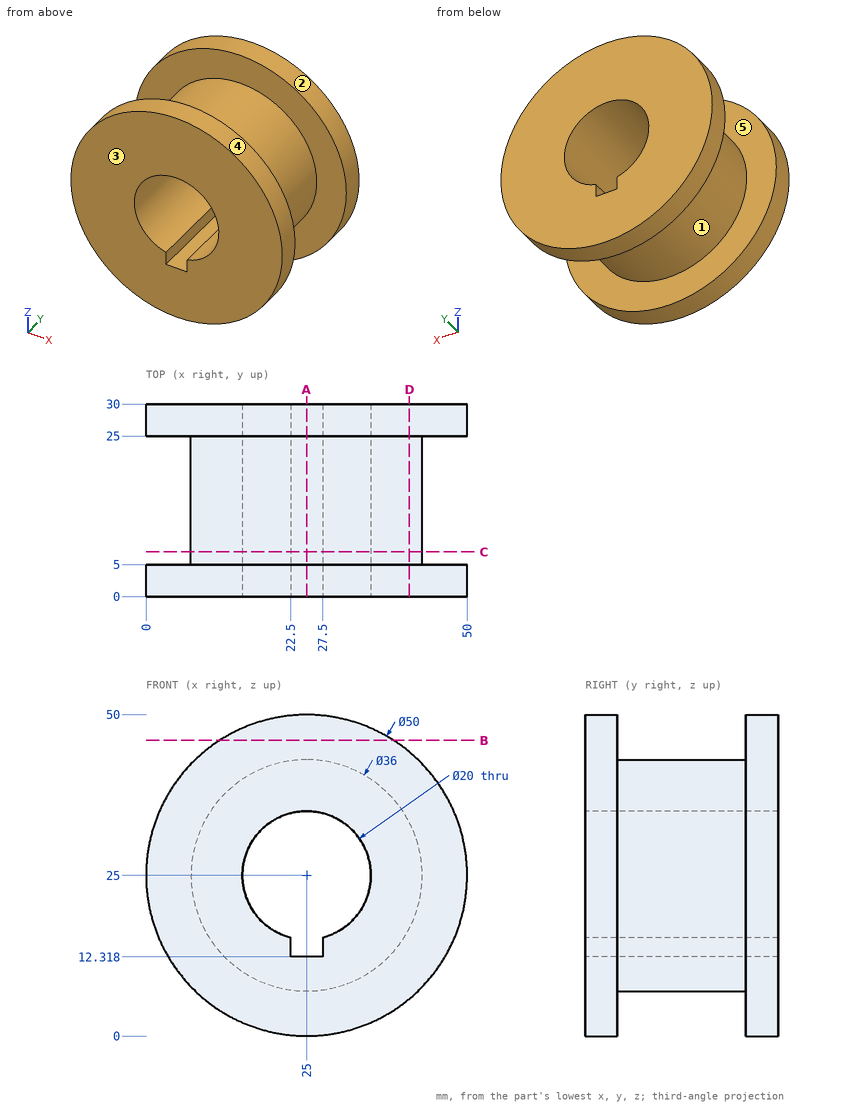
The figure shows three views and two pictorial views of one solid part (mm, origin at its lowest corner). Answer the questions. A direction names the side the tool comes from. Coordinates: 2 decimals unless noted, no trailing zeros. Order: outer loops, then holes, each group sorted by start corner. A loop starts at its lowest first (then second) coordinate and runs counter-clockwise, first axis right, second up.
Q1. A cutting plane is placed at C-C, the plane y = 7. Write down the section's boundary in (x, z).
Q2. A cutting plane is placed at B-B, the plane z = 46. Write down the section's boundary in (x, y) (1 decimal), and give its area (3 significant figures).
Q3. A cutting plane is placed at D-D, the plane x = 41. Write down the section's boundary in (y, z).
Q4. Given P1, Ø3, axis at y = 18, z = 26.5, coming from the -X side; P2, Ø2, axis at x = 24, y = 17, coming from the +Z side; P3, Ø6, axis at x = 40, y = 11, coming from the +Z side (1 decimal), each flat-ended and moving along its own axis, determine where each tip first touches the part or whether it passes through.
Q5. Consider line 1 (X direction, y = 21.75, z = 25); line 2 (Y direction, x = 13.5, z = 47); line 3 (X direction, y = 17.75, z = 31). Determine where each line is inside the solid, lowest interval first.
Q6. For a pull along Y with two mould halves and no side action, classify the marked faces 3, 4 and 5 as pulls with the +Y half, pulls with the -Y half, needs draft (parallel to the pull), parting line crosses it, or undercut.
Q7. A cutting plane is placed at A-A, the plane x = 25. Write down the section's boundary in (y, z).
Q8. Which of the six approach directions +Z, -Z, +X, -X, +Y, -Y give full straight-line access (tool end or side, diameter ignored) to the marked faces 1 and 2?
Answers follow:
1. outline: circle Ø36 at (25, 25); hole (22.5, 12.32) - (27.5, 12.32) - (27.5, 15.32) arc R10 ccw (long way) to (22.5, 15.32) - close
2. outline: (11.4, 0) - (38.6, 0) - (38.6, 5) - (11.4, 5) - close; (11.4, 25) - (38.6, 25) - (38.6, 30) - (11.4, 30) - close
2. area: 271 mm2
3. outline: (0, 5.79) - (5, 5.79) - (5, 16.75) - (25, 16.75) - (25, 5.79) - (30, 5.79) - (30, 44.21) - (25, 44.21) - (25, 33.25) - (5, 33.25) - (5, 44.21) - (0, 44.21) - close
4. P1: stops at x = 7
4. P2: stops at z = 43
4. P3: stops at z = 38.4
5. line 1: x = 7 to 15, 35 to 43
5. line 2: y = 0 to 5, 25 to 30
5. line 3: x = 8.03 to 17, 33 to 41.97
6. face 3: pulls with the -Y half
6. face 4: needs draft
6. face 5: undercut
7. outline: (0, 0) - (5, 0) - (5, 7) - (25, 7) - (25, 0) - (30, 0) - (30, 12.32) - (0, 12.32) - close; (0, 35) - (30, 35) - (30, 50) - (25, 50) - (25, 43) - (5, 43) - (5, 50) - (0, 50) - close
8. face 1: none
8. face 2: +Y, -Y
